Here's how the part is built. I have some questions about the finished solid (model axes, mm). A direction names the side the tool comes from. Round coordinates to 2 decimals unless told otherwise and drop trailing zeros. Loops run counter-clockwise (first coordinate to the right, second up) from the corner with the lowest first, then second, coordinate; pieces in that order, holes last. Notation, with made-up numbers: M 47,88.5 L 103,88.5 A22 cw 103,113.5 Z; hole C 26.25,64.5 d9. An arc over 180 degrees is marked long. Answer as CSV lines item,"result".
```python
from build123d import *

# Parameters (mm, degrees)
SKETCH1_R           = 30
BOSS_EXTRUDE1_DEPTH = 20
SKETCH2_R           = 8
BOSS_EXTRUDE2_DEPTH = 620
SKETCH3_R           = 30
BOSS_EXTRUDE3_DEPTH = 20


with BuildPart() as part:
    # Sketch1 → Boss-Extrude1 (new body)
    with BuildSketch(Plane.XY):
        Polygon((76.388888889, 0), (-76.388888889, 0), (-76.388888889, -5), (-100, -5), (-100, 15), (-68, 15), (-68, 45), (-100, 45), (-100, 245), (100, 245), (100, 45), (68, 45), (68, 15), (100, 15), (100, -5), (76.388888889, -5), align=None)
        with Locations((0, 145)):
            Circle(SKETCH1_R, mode=Mode.SUBTRACT)
    extrude(amount=BOSS_EXTRUDE1_DEPTH)

    # Sketch2 → Boss-Extrude2 (add)
    with BuildSketch(Plane.XY.offset(20)):
        with Locations(Location((-84, 229, 0), (0, 0, 180))):
            Circle(SKETCH2_R)
        with Locations(Location((84, 229, 0), (0, 0, 180))):
            Circle(SKETCH2_R)
        with Locations(Location((84, 61, 0), (0, 0, 180))):
            Circle(SKETCH2_R)
        with Locations(Location((-84, 61, 0), (0, 0, 180))):
            Circle(SKETCH2_R)
    extrude(amount=BOSS_EXTRUDE2_DEPTH)

    # Sketch3 → Boss-Extrude3 (add)
    with BuildSketch(Plane.XY.offset(640)):
        Polygon((76.388888889, 0), (-76.388888889, 0), (-76.388888889, -5), (-100, -5), (-100, 15), (-68, 15), (-68, 45), (-100, 45), (-100, 245), (100, 245), (100, 45), (68, 45), (68, 15), (100, 15), (100, -5), (76.388888889, -5), align=None)
        with Locations((0, 145)):
            Circle(SKETCH3_R, mode=Mode.SUBTRACT)
    extrude(amount=BOSS_EXTRUDE3_DEPTH)


solid = part.part
```
1. I want a section at C-C, the plane y = 102. Please give me the cut outline in (x, z).
Evaluation:
outline,"M -100,0 L 100,0 L 100,20 L -100,20 Z; M -100,640 L 100,640 L 100,660 L -100,660 Z"
2. Which directions (+Z, -Z, +X, -X, +Y, -Y) give clear straight access to the entire face, cutting with the end or side of a thin tool? Please do faces 1 (the flat face through (1, 0, 10)), 2 (the flat face through (84, 45, 650)), 3 (the cylindrical face through (-82.959, 53.068, 325.66)), 4 (the flat face through (-84, 45, 10)).
Evaluation:
face 1,"+Z, -Z, -Y"
face 2,"+Z, -Z, +X"
face 3,"none"
face 4,"+Z, -Z, -X"
3. I want a section at A-A, the plane x = 0. Please give me the cut outline in (y, z), and give its area (3 significant figures).
Evaluation:
outline,"M 0,0 L 115,0 L 115,20 L 0,20 Z; M 0,640 L 115,640 L 115,660 L 0,660 Z; M 175,0 L 245,0 L 245,20 L 175,20 Z; M 175,640 L 245,640 L 245,660 L 175,660 Z"
area,"7,400 mm²"
4. I want a section at D-D, the plane x = -46. Please give me the cut outline in (y, z).
Evaluation:
outline,"M 0,0 L 245,0 L 245,20 L 0,20 Z; M 0,640 L 245,640 L 245,660 L 0,660 Z"
5. We'd pull the mould along Y, two halves only. Please class faces 5 (the flat face through (84, 45, 10)), 6 (the flat face through (88, -5, 650)), 7 (the flat face through (100, 146, 10)), 8 (the flat face through (-1, 245, 10)): pulls with the +Y half, pulls with the -Y half, needs draft (parallel to the pull), parting line crosses it, or undercut.
Evaluation:
face 5,"undercut"
face 6,"pulls with the -Y half"
face 7,"needs draft"
face 8,"pulls with the +Y half"
6. If I drill on line 1 (Z direction, x = -19, y = 106); line 2 (Y direction, x = 0, z = 6); line 3 (Y direction, x = -85, z = 554.5), over which ranges is the centre line in solid material (lowest first)? Write a range as [from, to].
Evaluation:
line 1,"z = [0, 20], [640, 660]"
line 2,"y = [0, 115], [175, 245]"
line 3,"y = [53.06, 68.94], [221.06, 236.94]"
7. I want a section at B-B, the plane y = 145. Please give me the cut outline in (x, z).
Evaluation:
outline,"M -100,0 L -30,0 L -30,20 L -100,20 Z; M -100,640 L -30,640 L -30,660 L -100,660 Z; M 30,0 L 100,0 L 100,20 L 30,20 Z; M 30,640 L 100,640 L 100,660 L 30,660 Z"
8. For P1, Ø16, axis at x = 2, z = 11.5, coming from the -Y side; P2, Ø22, axis at y = 32, z = 651, coming from the +X side; P3, Ø1.5, axis at x = 4.5, y = 82.5, coming from the -Z side, each with a flat end and sliding along its axis, tell me the tip position at first contact or that it passes through.
Evaluation:
P1,"stops at y = 0"
P2,"stops at x = 68"
P3,"stops at z = 0"
